Could you check a few things on this model? Use its own coordinates, in mm. Face numbers are marked on the shaded views. A direction names the side the tool comes from. Round coordinates to 2 decimals unless told otherwise and drop trailing zeros. Write each loop counter-clockwise with the first axis right and the second up, starting at its lowest first coordinate (ties: lowest second). Pieces come first, ordered by that corner, then holes. Notation, with made-up numbers: (7.5, 32) -> (17.5, 32) arc R21 cw to (17.5, 67) -> close; hole circle Ø2 at (16, 9.5). An arc over 180 degrees is marked (long way). One line per question, with ' | ' between items. Start each with the question number.
1. Imagine slicing it at D-D, the plane z = 2. List the corners of the cut face in (x, y) for me, and give its area (3 significant figures).
2. If I drill on line 1 along X through (y, z) = (31.5, 8.89) (3 decimals); line 2 along X through (y, z) = (41, 14.5); line 3 along X through (y, z) = (36, 16), over which ranges is the centre line in solid material (lowest first)? Write a range as [from, to].
3. For pin 1 Ø6 at (y, z) = (42, 8) entering from +X; pin 2 Ø4 at (y, z) = (42, 3) entering from -X; pin 3 Ø9 at (x, z) = (-11, 12.5) entering from -Y, each with a flat end and sliding along its axis, tell me the tip position at first contact or that it passes through.
4. Imagine slicing it at C-C, the plane x = -10.16. List the corners of the cut face in (y, z) for me.
5. For the marked faces 1, 2 and 3, which set-ups out of +Z, -Z, +X, -X, +Y, -Y let a thin tool reach every point of the face, with its end or its side?
6. Imagine slicing it at B-B, the plane y = 40.64. List the corners of the cut face in (x, z) for me, and give its area (3 significant figures).
7. Thinking about a two-plate mould opening in X: for the marked faces 4, 5 and 6, which applies, released by +X, released by -X, zero draft, split by the parting line, or undercut?
8. Imagine slicing it at A-A, the plane z = 8.89. List the corners of the cut face in (x, y) for me, and give its area (3 significant figures).
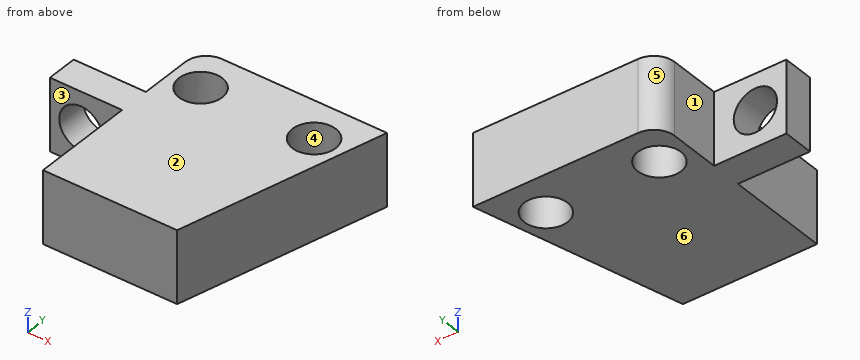
from build123d import *

# Parameters (mm, degrees)
SKETCH2_R           = 2.667
BOSS_EXTRUDE1_DEPTH = 8.89
SKETCH3_R           = 2.667
CUT_EXTRUDE1_DEPTH  = 30.566734686
FILLET1_R           = 2.54
SCALE1_SCALE        = 2


with BuildPart() as part:
    # Sketch2 → Boss-Extrude1 (new body)
    with BuildSketch(Plane.XY):
        Polygon((0, 0), (0, 12.7), (-8.89, 12.7), (-8.89, 16.51), (0, 16.51), (0, 25.4), (22.86, 25.4), (16.51, 0), align=None)
        with Locations((3.81, 20.32)):
            Circle(SKETCH2_R, mode=Mode.SUBTRACT)
        with Locations((17.78, 20.32)):
            Circle(SKETCH2_R, mode=Mode.SUBTRACT)
    extrude(amount=BOSS_EXTRUDE1_DEPTH)

    # Sketch3 → Cut-Extrude1 (cut, through all)
    with BuildSketch(Plane(origin=(0, 16.51, 0), x_dir=(1, 0, 0), z_dir=(0, 1, 0))):
        with Locations(Location((-5.08, -4.445, 0), (0, 0, 270))):
            Circle(SKETCH3_R)
    extrude(amount=-CUT_EXTRUDE1_DEPTH, mode=Mode.SUBTRACT)

    # Fillet1
    fillet1_edges = [part.edges().sort_by_distance(p)[0] for p in [
        (0, 25.4, 4.445),
    ]]
    fillet(fillet1_edges, radius=FILLET1_R)


with BuildPart() as part_1:
    # Scale1: scaled about (0, 0, 0)
    add(part.part.scale(SCALE1_SCALE))


solid = part_1.part
Geometry results:
1) outline: (-17.78, 25.4) -> (0, 25.4) -> (0, 0) -> (33.02, 0) -> (45.72, 50.8) -> (5.08, 50.8) arc R5.08 ccw to (0, 45.72) -> (0, 33.02) -> (-17.78, 33.02) -> close; hole circle Ø10.67 at (7.62, 40.64); hole circle Ø10.67 at (35.56, 40.64) | area: 1,950 mm2
2) line 1: x = [-17.78, -15.494], [-4.826, 40.895] | line 2: x = [0, 2.3], [12.94, 30.24], [40.88, 43.27] | line 3: x = [0, 4.99], [10.25, 32.93], [38.19, 42.02]
3) pin 1: stops at x = 44.27 | pin 2: stops at x = 0 | pin 3: stops at y = 25.4
4) outline: (25.4, 0) -> (33.02, 0) -> (33.02, 3.56) -> (25.4, 3.56) -> close; (25.4, 14.22) -> (33.02, 14.22) -> (33.02, 17.78) -> (25.4, 17.78) -> close
5) face 1: +Z, -Z, -X, +Y | face 2: +Z, +X, -X, +Y, -Y | face 3: +Z, -Z, -X, -Y
6) outline: (0, 0) -> (2.29, 0) -> (2.29, 17.78) -> (0, 17.78) -> close; (12.95, 0) -> (30.23, 0) -> (30.23, 17.78) -> (12.95, 17.78) -> close; (40.89, 0) -> (43.18, 0) -> (43.18, 17.78) -> (40.89, 17.78) -> close | area: 388 mm2
7) face 4: undercut | face 5: released by -X | face 6: zero draft
8) outline: (-17.78, 25.4) -> (-15.49, 25.4) -> (-15.49, 33.02) -> (-17.78, 33.02) -> close; (-4.83, 25.4) -> (0, 25.4) -> (0, 0) -> (33.02, 0) -> (45.72, 50.8) -> (5.08, 50.8) arc R5.08 ccw to (0, 45.72) -> (0, 33.02) -> (-4.83, 33.02) -> close; hole circle Ø10.67 at (7.62, 40.64); hole circle Ø10.67 at (35.56, 40.64) | area: 1,870 mm2
